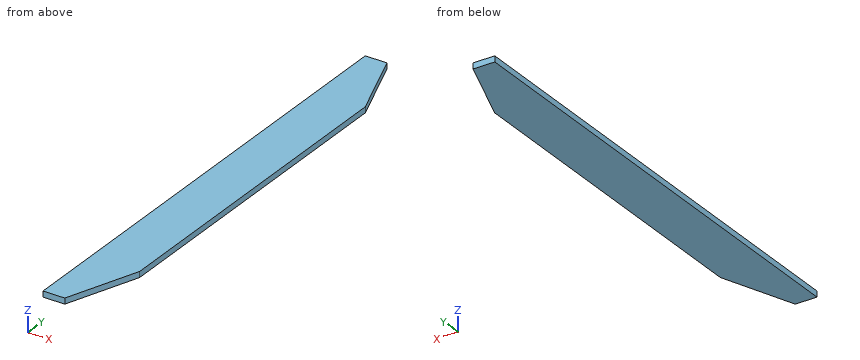
from build123d import *

# Parameters (mm, degrees)
BOSS_EXTRUDE1_DEPTH = 6


with BuildPart() as part:
    # Sketch1 → Boss-Extrude1 (new, symmetric)
    with BuildSketch(Plane.XY):
        Polygon((0, -500), (0, 500), (45, 500), (100, 350), (100, -350), (45, -500), align=None)
    extrude(amount=BOSS_EXTRUDE1_DEPTH, both=True)


solid = part.part
Verification items for the finished model (mm, model axes). Coordinates: 2 decimals unless noted, no trailing zeros. Order: outer loops, then holes, each group sorted by start corner. A loop starts at its lowest first (then second) coordinate and runs counter-clockwise, first axis right, second up.
Item 1: Depth check by flat-ended pin: pin 1 (5 mm diameter, centred on y = 222, z = -2, fed in from -X). Enter the tip coordinate at first touch or a pass-through.
Filled in:
pin 1: stops at x = 0
Item 2: Material ranges on L1, parallel to X at y = 433.5, z = -4.75, recorded low to high.
Filled in:
L1: x = 0 to 69.38
Item 3: Section check B-B, the plane y = -423.5. Enter the section's corners in (x, z), then the cut area to 3 significant figures.
Filled in:
outline: (0, -6) - (73.05, -6) - (73.05, 6) - (0, 6) - close
area: 877 mm2
Item 4: Section check C-C, the plane x = 78. Enter the section's corners in (y, z), then the cut area to 3 significant figures.
Filled in:
outline: (-410, -6) - (410, -6) - (410, 6) - (-410, 6) - close
area: 9,840 mm2
Item 5: Section check A-A, the plane z = -0.25. Enter the section's corners in (x, y).
Filled in:
outline: (0, -500) - (45, -500) - (100, -350) - (100, 350) - (45, 500) - (0, 500) - close
